```python
from build123d import *

# Parameters (mm, degrees)
CONECUT_DEPTH      = 27.521877713
CONECUT_DEPTH_BACK = 27.521877713


with BuildPart() as part:
    # Body: sweep along a path in Sketch2
    with BuildLine(Plane.XY) as body_path:
        Line((22, 2.5), (0, 2.5))
        ThreePointArc((0, 2.5), (-1.229728386, 2.730698436), (-2.292225201, 3.391420912))
        ThreePointArc((-2.292225201, 3.391420912), (-10, 0), (-2.292225201, -3.391420912))
        ThreePointArc((-2.292225201, -3.391420912), (-1.229728386, -2.730698436), (0, -2.5))
        Line((0, -2.5), (26, -2.5))
    # Sketch1 → Body (sweep)
    with BuildSketch(Plane(origin=(22, 0, 0), x_dir=(0, 0, -1), z_dir=(1, 0, 0))):
        with BuildLine():
            Line((-2.4999992, 0.002), (2.4999992, 0.002))
            ThreePointArc((2.4999992, 0.002), (0, 2.5), (-2.4999992, 0.002))
        make_face()
    sweep(path=body_path.line)

    # Sketch3 → ConeCut (cut, two sides: drawn at the far end of the back side and taken through both)
    with BuildSketch(Plane.XY.offset(-CONECUT_DEPTH_BACK)):
        Polygon((22, 1.251), (20.210475082, 2.51), (26.01, 2.51), (26.01, -2.51), (24.210475082, -2.51), (26, -1.251), (24.204873421, 0), (20.204873421, 0), align=None)
    extrude(amount=CONECUT_DEPTH + CONECUT_DEPTH_BACK, mode=Mode.SUBTRACT)


solid = part.part
```
Build history of the part. All positions in model axes, mm. A direction names the side the tool comes from. Round coordinates to 2 decimals unless told otherwise and drop trailing zeros. Answer as CSV lines item,"result".
Q1. Drill centre lines: probe 1 along Y at (x, z) = (23, 0.1); probe 2 along Y at (x, z) = (-5.4, -1.2); probe 3 along Y at (x, z) = (-5.4, -0.8). Where is each one in solid material? Low to high. Write a range as [from, to].
Report:
probe 1,"y = [-2.5, 0]"
probe 2,"y = [-4.29, -2.1], [2.1, 4.29]"
probe 3,"y = [-4.47, -2.1], [2.1, 4.47]"
Q2. Drop flat-ended pins along their axis: pin 1 (3.5 mm diameter, centred on x = -5.4, y = 0, fed in from -Z); pin 2 (1.5 mm diameter, centred on x = 4.5, z = 1, fed in from -Y); pin 3 (5 mm diameter, centred on x = -2, y = 1, fed in from -Z). Give the stop position or say it passes through.
Report:
pin 1,"passes through"
pin 2,"stops at y = -2.49"
pin 3,"stops at z = -2.5"
Q3. Pull direction Y, two halves, no side cores. Call faces 1 (the cylindrical face through (-7.5, 0.1, 0)), 2 (the flat face through (21.091, 0.618, -0.035)), 3 (the flat face through (25.12, -0.64, -0.03)), 4 (the cylindrical face through (13.2, -2.5, 0.1)): +Y half, -Y half, draft (parallel to the pull), parting line (faces both ways), or undercut.
Report:
face 1,"undercut"
face 2,"undercut"
face 3,"+Y half"
face 4,"-Y half"
Q4. Tool access for faces 5 (the flat face through (25.297, -1.745, -0.03)), 6 (the cylindrical face through (10.8, 2.5, 0.1)): list every direction of +Z, -Z, +X, -X, +Y, -Y with a clear straight run to the whole face (end or side of a thin tool).
Report:
face 5,"+Z, -Z, +X, -Y"
face 6,"+X, +Y"
